Design review of the part built by this model. Coordinates are the model's own, in mm. Face numbers are marked on the shaded views. A direction names the side the tool comes from. Give positions to 0.01 mm unless a question says otherwise; leave off trailing zeros. Loops run counter-clockwise (first coordinate to the right, second up) from the corner with the lowest first, then second, coordinate; pieces in that order, holes last. Notation, with made-up numbers: (59, 28) - (109, 28) arc R29 cw to (109, 52) - close; hole circle Ø6 at (2, -15). An arc over 180 degrees is marked (long way). Put each result on its own line as item: value. Start each with the question number.
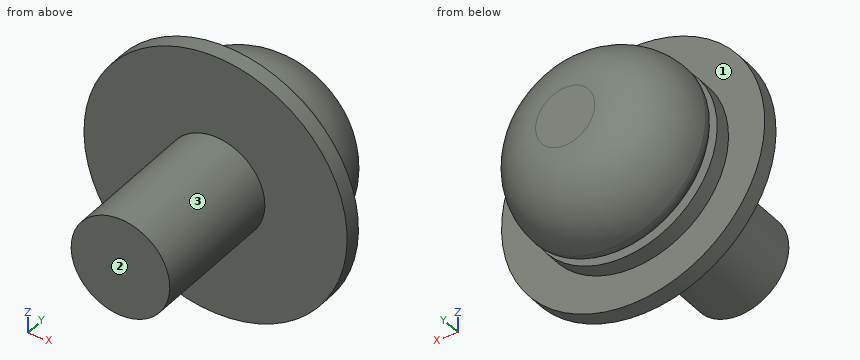
```python
from build123d import *


with BuildPart() as part:
    # Sketch1 → Revolve1 (revolve)
    with BuildSketch(Plane(origin=(0, 0, 0), x_dir=(0, 0, -1), z_dir=(1, 0, 0)), mode=Mode.PRIVATE) as revolve1_sk:
        with BuildLine():
            Line((0, -4.2), (-1.5, -4.2))
            Line((-1.5, -4.2), (-1.5, 0))
            Line((-1.5, 0), (-4, 0))
            Line((-4, 0), (-4, 0.5))
            Line((-4, 0.5), (-2.9, 0.5))
            Line((-2.9, 0.5), (-2.9, 1))
            Line((-2.9, 1), (-2.4, 1))
            ThreePointArc((-2.4, 1), (-2.753553391, 1.146446609), (-2.9, 1.5))
            ThreePointArc((-2.9, 1.5), (-2.314213562, 2.914213562), (-0.9, 3.5))
            Line((-0.9, 3.5), (0, 3.5))
            Line((0, 3.5), (0, -4.2))
        make_face()
    revolve(revolve1_sk.sketch.rotate(Axis((0, 3.5, 0), (0, -1, 0)), 180), axis=Axis((0, 3.5, 0), (0, -1, 0)))


solid = part.part
```
Item 1: For L1, parallel to Y at x = 0.75, z = -3.5; L2, parallel to Y at x = -2, z = -0.5; L3, parallel to Z at x = 0.75, y = -0.5, list the stretches that pass through material, from the lowest coordinate up. Write a range as from..to.
Item 2: Consider section C-C (z = 3.5). State the section outline as (x, y) points, plus the area to 3 significant figures.
Item 3: Machinability: for the marked faces 1, 2 and 3, which of the approach directions +Z, -Z, +X, -X, +Y, -Y give a long, thin tool a straight path to every point of the face, cutting with its end or side? Answer none if there is none.
Item 4: Consider section A-A (y = 0.75). State the section outline as (x, z) points.
Item 5: Consider section B-B (x = 3.25). State the section outline as (y, z) points.
Item 6: For P1, Ø2, axis at x = -3, z = -3, coming from the -Y side; P2, Ø4, axis at x = -1.5, y = -3, coming from the -Z side, all flat-tipped, find the tip position at first contact; note any pin that passes through.
Geometry says:
1. L1: y = 0..0.5
1. L2: y = 0..3.13
1. L3: z = -1.3..1.3
2. outline: (-1.94, 0) - (1.94, 0) - (1.94, 0.5) - (-1.94, 0.5) - close
2. area: 1.94 mm2
3. face 1: +Y
3. face 2: +Z, -Z, +X, -X, -Y
3. face 3: -Y
4. outline: circle Ø5.8 at (0, 0)
5. outline: (0, -2.33) - (0.5, -2.33) - (0.5, 2.33) - (0, 2.33) - close
6. P1: stops at y = 0
6. P2: stops at z = -1.5
